```python
from build123d import *

# Parameters (mm, degrees)
EXTRUDE_1_DEPTH     = 1550
SKETCH_2_R          = 12
CUT_EXTRUDE_1_DEPTH = 10
SKETCH_3_R          = 16.065065839
SKETCH_3_R_2        = 15.441664685
EXTRUDE_2_DEPTH     = 5
SKETCH_4_W          = 38
SKETCH_4_H          = 630.491026123
EXTRUDE_3_DEPTH     = 5
SKETCH_5_R          = 10
CUT_EXTRUDE_2_DEPTH = 10


with BuildPart() as part:
    # 草图1 → 凸台-拉伸1 (new body)
    with BuildSketch(Plane(origin=(0, 0, 0), x_dir=(1, 0, 0), z_dir=(0, 1, 0))):
        with BuildLine():
            Line((-19, -12.278106509), (19, -12.278106509))
            ThreePointArc((19, -12.278106509), (23.242640687, -10.520747196), (25, -6.278106509))
            Line((25, -6.278106509), (25, 31.721893491))
            ThreePointArc((25, 31.721893491), (23.242640687, 35.964534178), (19, 37.721893491))
            Line((19, 37.721893491), (-19, 37.721893491))
            ThreePointArc((-19, 37.721893491), (-23.242640687, 35.964534178), (-25, 31.721893491))
            Line((-25, 31.721893491), (-25, -6.278106509))
            ThreePointArc((-25, -6.278106509), (-23.242640687, -10.520747196), (-19, -12.278106509))
        make_face()
        with BuildLine():
            Line((-19, -7.278106509), (19, -7.278106509))
            ThreePointArc((19, -7.278106509), (19.707106781, -6.98521329), (20, -6.278106509))
            Line((20, -6.278106509), (20, 31.721893491))
            ThreePointArc((20, 31.721893491), (19.707106781, 32.429000272), (19, 32.721893491))
            Line((19, 32.721893491), (-19, 32.721893491))
            ThreePointArc((-19, 32.721893491), (-19.707106781, 32.429000272), (-20, 31.721893491))
            Line((-20, 31.721893491), (-20, -6.278106509))
            ThreePointArc((-20, -6.278106509), (-19.707106781, -6.98521329), (-19, -7.278106509))
        make_face(mode=Mode.SUBTRACT)
    extrude(amount=EXTRUDE_1_DEPTH)

    # 草图2 → 切除-拉伸1 (cut)
    with BuildSketch(Plane(origin=(25, 0, 0), x_dir=(0, 0, -1), z_dir=(1, 0, 0))):
        with Locations((12.721893491, 1527.5)):
            Circle(SKETCH_2_R)
        with Locations((12.721893491, 1482.5)):
            Circle(SKETCH_2_R)
        with Locations((12.721893491, 1437.5)):
            Circle(SKETCH_2_R)
        with Locations((12.721893491, 1392.5)):
            Circle(SKETCH_2_R)
        with Locations((12.721893491, 1347.5)):
            Circle(SKETCH_2_R)
        with Locations((12.721893491, 1302.5)):
            Circle(SKETCH_2_R)
        with Locations((12.721893491, 1257.5)):
            Circle(SKETCH_2_R)
        with Locations((12.721893491, 1212.5)):
            Circle(SKETCH_2_R)
        with Locations((12.721893491, 1167.5)):
            Circle(SKETCH_2_R)
        with Locations((12.721893491, 1122.5)):
            Circle(SKETCH_2_R)
        with Locations((12.721893491, 1077.5)):
            Circle(SKETCH_2_R)
        with Locations((12.721893491, 1032.5)):
            Circle(SKETCH_2_R)
        with Locations((12.721893491, 987.5)):
            Circle(SKETCH_2_R)
        with Locations((12.721893491, 942.5)):
            Circle(SKETCH_2_R)
        with Locations((12.721893491, 897.5)):
            Circle(SKETCH_2_R)
    extrude(amount=-CUT_EXTRUDE_1_DEPTH, mode=Mode.SUBTRACT)

    # 草图3 → 凸台-拉伸2 (add)
    with BuildSketch(Plane(origin=(25, 0, 0), x_dir=(0, 0, -1), z_dir=(1, 0, 0))):
        with Locations((12.721893491, 897.5)):
            Circle(SKETCH_3_R)
        with Locations((12.721893491, 1527.5)):
            Circle(SKETCH_3_R_2)
    extrude(amount=-EXTRUDE_2_DEPTH)

    # 草图4 → 凸台-拉伸3 (add)
    with BuildSketch(Plane(origin=(25, 0, 0), x_dir=(0, 0, -1), z_dir=(1, 0, 0))):
        with Locations((12.721893491, 1196.647134408)):
            Rectangle(SKETCH_4_W, SKETCH_4_H)
    extrude(amount=-EXTRUDE_3_DEPTH)

    # 草图5 → 切除-拉伸2 (cut)
    with BuildSketch(Plane(origin=(25, 0, 0), x_dir=(0, 0, -1), z_dir=(1, 0, 0))):
        with Locations((12.721893491, 1490)):
            Circle(SKETCH_5_R)
        with Locations((12.721893491, 1445)):
            Circle(SKETCH_5_R)
        with Locations((12.721893491, 1400)):
            Circle(SKETCH_5_R)
        with Locations((12.721893491, 1355)):
            Circle(SKETCH_5_R)
        with Locations((12.721893491, 1310)):
            Circle(SKETCH_5_R)
        with Locations((12.721893491, 1265)):
            Circle(SKETCH_5_R)
        with Locations((12.721893491, 1220)):
            Circle(SKETCH_5_R)
        with Locations((12.721893491, 1175)):
            Circle(SKETCH_5_R)
        with Locations((12.721893491, 1130)):
            Circle(SKETCH_5_R)
        with Locations((12.721893491, 1085)):
            Circle(SKETCH_5_R)
        with Locations((12.721893491, 1040)):
            Circle(SKETCH_5_R)
        with Locations((12.721893491, 995)):
            Circle(SKETCH_5_R)
        with Locations((12.721893491, 950)):
            Circle(SKETCH_5_R)
        with Locations((12.721893491, 905)):
            Circle(SKETCH_5_R)
        with Locations((12.721893491, 860)):
            Circle(SKETCH_5_R)
        with Locations((12.721893491, 815)):
            Circle(SKETCH_5_R)
        with Locations((12.721893491, 770)):
            Circle(SKETCH_5_R)
        with Locations((12.721893491, 725)):
            Circle(SKETCH_5_R)
        with Locations((12.721893491, 680)):
            Circle(SKETCH_5_R)
        with Locations((12.721893491, 635)):
            Circle(SKETCH_5_R)
        with Locations((12.721893491, 590)):
            Circle(SKETCH_5_R)
        with Locations((12.721893491, 545)):
            Circle(SKETCH_5_R)
        with Locations((12.721893491, 500)):
            Circle(SKETCH_5_R)
        with Locations((12.721893491, 455)):
            Circle(SKETCH_5_R)
        with Locations((12.721893491, 410)):
            Circle(SKETCH_5_R)
        with Locations((12.721893491, 365)):
            Circle(SKETCH_5_R)
        with Locations((12.721893491, 320)):
            Circle(SKETCH_5_R)
        with Locations((12.721893491, 275)):
            Circle(SKETCH_5_R)
        with Locations((12.721893491, 230)):
            Circle(SKETCH_5_R)
        with Locations((12.721893491, 185)):
            Circle(SKETCH_5_R)
        with Locations((12.721893491, 140)):
            Circle(SKETCH_5_R)
    extrude(amount=-CUT_EXTRUDE_2_DEPTH, mode=Mode.SUBTRACT)


solid = part.part
```
Work out the finished part from the listing and answer in its coordinate system (mm). A direction names the side the tool comes from. Give positions to 0.01 mm unless a question says otherwise; leave off trailing zeros. Write each loop counter-clockwise with the first axis right and the second up, starting at its lowest first coordinate (ties: lowest second). Pieces come first, ordered by that corner, then holes. Notation, with made-up numbers: (55, -1) -> (94, -1) arc R21 ccw to (94, 4) -> close; hole circle Ø5 at (-7.5, 83.25). An arc over 180 degrees is marked (long way). Write item = value, one per line.
Q1. Consider line 1 along Z through (x, y) = (-12.5, 929.5); line 2 along X through (y, z) = (1133.5, -22.5); line 3 along X through (y, z) = (959.5, -10). Determine where each line is inside the solid, lowest interval first.
Computed values:
line_1 = -37.72 to -32.72, 7.28 to 12.28
line_2 = -25 to -20, 20 to 25
line_3 = -25 to -20
Q2. Section A-A on x = -7.5 is taken. Determine the outline of the cut face in (y, z), and give its area (3 significant figures).
Computed values:
outline = (0, -37.72) -> (1550, -37.72) -> (1550, -32.72) -> (0, -32.72) -> close; (0, 7.28) -> (1550, 7.28) -> (1550, 12.28) -> (0, 12.28) -> close
area = 15,500 mm^2
Q3. Flat-ended cylindrical pins translate along their axes: pin 1 Ø18 at (y, z) = (320, -12.72) entering from +X; pin 2 Ø8 at (x, z) = (13, -10.5) entering from +Y. Find the tip coordinate at first contact, or state that the pin passes through.
Computed values:
pin_1 = -20
pin_2 = through
Q4. A tool of negligible diameter and unlimited length cuts with its end or side. For faces 5 (the flat face through (-20, 764, -13)), 6 (the flat face through (25, 764, -4)), from which of +Z, -Z, +X, -X, +Y, -Y can it reach the whole face along a straight path? Write none if from no direction.
Computed values:
face_5 = +Y, -Y
face_6 = +Z, -Z, +X, +Y, -Y
Q5. For a pull along Z with two mould halves and no side action, classify faces 1 (the flat face through (0, 764, -32.722)), 2 (the flat face through (-23, 1550, -13)), 3 (the flat face through (0, 764, 12.278)), 4 (the flat face through (0, 764, -37.722)) as pulls with the +Z half, pulls with the -Z half, needs draft (parallel to the pull), parting line crosses it, or undercut.
Computed values:
face_1 = undercut
face_2 = needs draft
face_3 = pulls with the +Z half
face_4 = pulls with the -Z half
